from build123d import *

# Parameters (mm, degrees)
PLATE_PROFILE_SKETCH_R      = 12
PROFILED_PLATE_20MM_DEPTH   = 20
BORE_CHAMFER_1_5X45DEG_SIZE = 1.5


with BuildPart() as part:
    # Plate Profile Sketch → Profiled Plate 20mm (new body)
    with BuildSketch(Plane(origin=(0, 0, 0), x_dir=(0, 0, -1), z_dir=(1, 0, 0))):
        with BuildLine():
            Line((41, 73), (41, 48.5))
            ThreePointArc((41, 48.5), (29, 36.5), (41, 24.5))
            Line((41, 24.5), (41, 0))
            Line((41, 0), (0, 0))
            Line((0, 0), (-41, 0))
            Line((-41, 0), (-41, 24.5))
            ThreePointArc((-41, 24.5), (-29, 36.5), (-41, 48.5))
            Line((-41, 48.5), (-41, 73))
            ThreePointArc((-41, 73), (0, 114), (41, 73))
        make_face()
        with Locations((0, 57)):
            Circle(PLATE_PROFILE_SKETCH_R, mode=Mode.SUBTRACT)
        with BuildLine():
            ThreePointArc((9.4, 25.713142743), (0, 31), (-9.4, 25.713142743))
            ThreePointArc((-9.4, 25.713142743), (-23, 20), (-9.4, 14.286857257))
            ThreePointArc((-9.4, 14.286857257), (0, 9), (9.4, 14.286857257))
            ThreePointArc((9.4, 14.286857257), (23, 20), (9.4, 25.713142743))
        make_face(mode=Mode.SUBTRACT)
        with BuildLine():
            ThreePointArc((28.578838325, 89.5), (0, 106), (-28.578838325, 89.5))
            ThreePointArc((-28.578838325, 89.5), (-26.382685902, 81.303847577), (-18.186533479, 83.5))
            ThreePointArc((-18.186533479, 83.5), (0, 94), (18.186533479, 83.5))
            ThreePointArc((18.186533479, 83.5), (26.382685902, 81.303847577), (28.578838325, 89.5))
        make_face(mode=Mode.SUBTRACT)
    extrude(amount=PROFILED_PLATE_20MM_DEPTH)

    # Bore Chamfer 1.5x45deg
    bore_chamfer_1_5x45deg_edges = [part.edges().sort_by_distance(p)[0] for p in [
        (0, 57, 12),
        (20, 57, 12),
    ]]
    chamfer(bore_chamfer_1_5x45deg_edges, length=BORE_CHAMFER_1_5X45DEG_SIZE)


solid = part.part
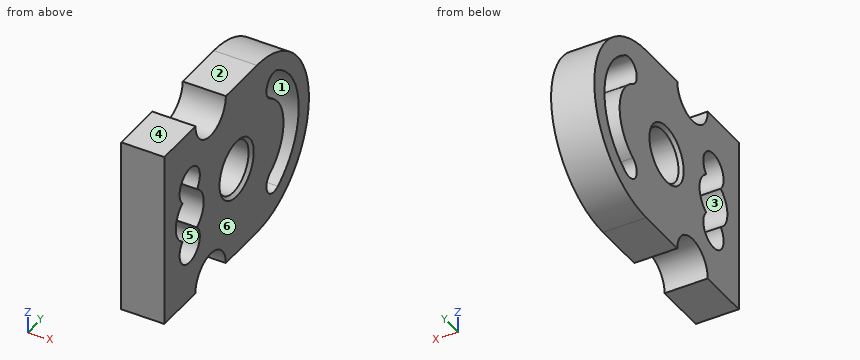
Build history of the part. All positions in model axes, mm. Face numbers are marked on the shaded views. A direction names the side the tool comes from. Coordinates: 2 decimals unless noted, no trailing zeros. Write each loop counter-clockwise with the first axis right and the second up, starting at its lowest first coordinate (ties: lowest second). Pieces come first, ordered by that corner, then holes. Notation, with made-up numbers: (42.5, 1) -> (92.5, 1) arc R29 cw to (92.5, 30) -> close; hole circle Ø8 at (75.5, -12.75). An arc over 180 degrees is marked (long way). Use CSV: the item, a comma, the result in double quotes. Start each with the question number.
Q1. Cut at A-A, the plane z = 0. List the corners of the cut face in (x, y), then the cut area to 3 significant figures.
Q2. Cut at D-D, the plane z = -15. List the corners of the cut face in (x, y), then the cut area to 3 significant figures.
Q3. Pull direction Z, two halves, no side cores. Call the marked faces 3, 4, 5 and 6: released by +Z, released by -Z, zero draft, split by the parting line, or undercut.
Q4. Flat gauge pins, fed straight in: pin 1 Ø6 at (y, z) = (96.5, 9.5) entering from +X; pin 2 Ø10 at (x, z) = (12, 4.5) entering from +Y; pin 3 Ø1 at (x, z) = (5.5, 26) entering from +Y. Where does each tip first touch, or does it go through?
Q5. Drill centre lines: probe 1 along Z at (x, y) = (9.25, 20); probe 2 along Y at (x, z) = (15, -15); probe 3 along Y at (x, z) = (15.25, 5). Where is each one in solid material? Low to high.
Q6. Cut at B-B, the plane x = 7.5. List the corners of the cut face in (y, z).
Q7. Cut at C-C, the plane y = 20. List the corners of the cut face in (x, z).
Q8. 3-axis set-ups, long thin cutter, end or side, ignore diameter. For the marked faces 1 and 2: which of +Z, -Z, +X, -X, +Y, -Y reach the whole face in a straight line?
Checked values:
1,outline,"(0, 0) -> (20, 0) -> (20, 9) -> (0, 9) -> close; (0, 31) -> (20, 31) -> (20, 43.5) -> (18.5, 45) -> (1.5, 45) -> (0, 43.5) -> close; (0, 70.5) -> (1.5, 69) -> (18.5, 69) -> (20, 70.5) -> (20, 94) -> (0, 94) -> close; (0, 106) -> (20, 106) -> (20, 114) -> (0, 114) -> close"
1,area,"1,120 mm²"
2,outline,"(0, 0) -> (20, 0) -> (20, 12) -> (0, 12) -> close; (0, 28) -> (20, 28) -> (20, 87.7) -> (0, 87.7) -> close; (0, 102.39) -> (20, 102.39) -> (20, 111.16) -> (0, 111.16) -> close"
2,area,"1,610 mm²"
3,face 3,"undercut"
3,face 4,"released by +Z"
3,face 5,"undercut"
3,face 6,"zero draft"
4,pin 1,"passes through"
4,pin 2,"stops at y = 114"
4,pin 3,"stops at y = 105.11"
5,probe 1,"z = -41 to -23, 23 to 41"
5,probe 2,"y = 0 to 12, 28 to 87.7, 102.39 to 111.16"
5,probe 3,"y = 0 to 10.2, 29.8 to 46.09, 67.91 to 93.4, 105.62 to 113.69"
6,outline,"(0, -41) -> (24.5, -41) arc R12 cw to (48.5, -41) -> (73, -41) arc R41 ccw to (73, 41) -> (48.5, 41) arc R12 cw to (24.5, 41) -> (0, 41) -> close; hole (14.29, -9.4) arc R8 ccw (long way) to (25.71, -9.4) arc R11 ccw to (25.71, 9.4) arc R8 ccw (long way) to (14.29, 9.4) arc R11 ccw to start; hole circle Ø24 at (57, 0); hole (83.5, -18.19) arc R6 ccw to (89.5, -28.58) arc R33 ccw to (89.5, 28.58) arc R6 ccw to (83.5, 18.19) arc R21 cw to start"
7,outline,"(0, -41) -> (20, -41) -> (20, -23) -> (0, -23) -> close; (0, 23) -> (20, 23) -> (20, 41) -> (0, 41) -> close"
8,face 1,"+X, -X"
8,face 2,"+Z, +X, -X, +Y, -Y"
